```python
from build123d import *

# Parameters (mm, degrees)
SKETCH1_W           = 550
SKETCH1_H           = 300
BOSS_EXTRUDE1_DEPTH = 200
SHELL1_T            = -1.5
SKETCH2_W           = 550
SKETCH2_H           = 300
BOSS_EXTRUDE2_DEPTH = 1
SKETCH3_W           = 530
SKETCH3_H           = 280
SKETCH3_W_2         = 526
SKETCH3_H_2         = 276
SKETCH3_W_3         = 24
SKETCH3_H_3         = 80
CUT_EXTRUDE1_DEPTH  = 0.5
SKETCH5_R           = 11
SKETCH5_W           = 92
SKETCH5_H           = 45
CUT_EXTRUDE2_DEPTH  = 0.5


with BuildPart() as part:
    # Sketch1 → Boss-Extrude1 (new body)
    with BuildSketch(Plane.XY):
        with Locations((275, 150)):
            Rectangle(SKETCH1_W, SKETCH1_H)
    extrude(amount=BOSS_EXTRUDE1_DEPTH)

    # Shell1
    shell1_openings = [part.faces().sort_by_distance(p)[0] for p in [
        (275, 150, 200),
    ]]
    offset(amount=SHELL1_T, openings=shell1_openings, kind=Kind.INTERSECTION)

    # Sketch2 → Boss-Extrude2 (add)
    with BuildSketch(Plane.XY.offset(200)):
        with Locations((275, 150)):
            Rectangle(SKETCH2_W, SKETCH2_H)
    extrude(amount=BOSS_EXTRUDE2_DEPTH)

    # Sketch3 → Cut-Extrude1 (cut)
    # profile 1 of 2: a face of its own
    with BuildSketch(Plane.XY.offset(201)):
        with Locations((275, 150)):
            Rectangle(SKETCH3_W, SKETCH3_H)
        with Locations((275, 150)):
            Rectangle(SKETCH3_W_2, SKETCH3_H_2, mode=Mode.SUBTRACT)
    # profile 2 of 2: a face of its own
    with BuildSketch(Plane.XY.offset(201)):
        with Locations((511, 150)):
            Rectangle(SKETCH3_W_3, SKETCH3_H_3)
    extrude(amount=-CUT_EXTRUDE1_DEPTH, mode=Mode.SUBTRACT)

    # Sketch5 → Cut-Extrude2 (cut)
    with BuildSketch(Plane(origin=(550, 0, 0), x_dir=(0, 0, -1), z_dir=(1, 0, 0))):
        with Locations((-143, 110)):
            Circle(SKETCH5_R)
        with Locations((-58, 110)):
            Circle(SKETCH5_R)
        with Locations((-100.5, 217.5)):
            Rectangle(SKETCH5_W, SKETCH5_H)
    extrude(amount=-CUT_EXTRUDE2_DEPTH, mode=Mode.SUBTRACT)


solid = part.part
```
The model under review builds one solid part; all positions refer to its coordinate system, in mm. A direction names the side the tool comes from. Round coordinates to 2 decimals unless told otherwise and drop trailing zeros. Write each loop counter-clockwise with the first axis right and the second up, starting at its lowest first coordinate (ties: lowest second). Pieces come first, ordered by that corner, then holes. Notation, with made-up numbers: (-2.75, 4) - (22.25, 4) arc R22 cw to (22.25, 29) - close; hole circle Ø4 at (18, 36.5). An arc over 180 degrees is marked (long way). Use one line per item in the form item = value.
Q1. For line 1 (Y direction, x = 549.8, z = 58); line 2 (Z direction, x = 52.5, y = 51.5); line 3 (X direction, y = 115, z = 127.5), list the stretches that pass through material, from the lowest coordinate up. Write a range as [from, to].
Answer key:
line_1 = [0, 99], [121, 195], [240, 300]
line_2 = [0, 1.5], [200, 201]
line_3 = [0, 1.5], [548.5, 550]
Q2. Draft analysis for pull direction Z (two halves, no side actions). For faces 1 (the flat face through (548.5, 148, 99)), 2 (the flat face through (192, 6, 201)), 3 (the flat face through (271, 152, 0)), state which applies: +Z half, -Z half, draft (parallel to the pull), parting line (faces both ways), or undercut.
Answer key:
face_1 = undercut
face_2 = +Z half
face_3 = -Z half
Q3. Consider section C-C (z = 171). State the section outline as (x, y) points.
Answer key:
outline = (0, 0) - (550, 0) - (550, 300) - (0, 300) - close; hole (1.5, 1.5) - (548.5, 1.5) - (548.5, 298.5) - (1.5, 298.5) - close
Q4. Insertion check: pin 1 Ø13 at (y, z) = (110, 143) entering from -X; pin 2 Ø13.5 at (y, z) = (227, 83.5) entering from +X. Each pin has a flat end and moves straight along its axis. Give the tip position at first contact, or say it passes through.
Answer key:
pin_1 = 0
pin_2 = 549.5
Q5. Tool access review of faces 4 (the flat face through (511, 151, 200.5)), 5 (the flat face through (0, 148, 99)), 6 (the flat face through (549.5, 218, 101)), 7 (the flat face through (271, 0, 99)), 8 (the flat face through (271, 298.5, 99)): name each direction out of +Z, -Z, +X, -X, +Y, -Y from which nothing blocks a thin tool from reaching the whole face with its end or side.
Answer key:
face_4 = +Z
face_5 = +Z, -Z, -X, +Y, -Y
face_6 = +X
face_7 = +Z, -Z, +X, -X, -Y
face_8 = none
Q6. Consider section A-A (z = 77). State the section outline as (x, y) points, and give its area (3 significant figures).
Answer key:
outline = (0, 0) - (550, 0) - (550, 195) - (549.5, 195) - (549.5, 240) - (550, 240) - (550, 300) - (0, 300) - close; hole (1.5, 1.5) - (548.5, 1.5) - (548.5, 298.5) - (1.5, 298.5) - close
area = 2,520 mm2
Q7. Consider section B-B (x = 221). State the section outline as (y, z) points, and give its area (3 significant figures).
Answer key:
outline = (0, 0) - (300, 0) - (300, 201) - (290, 201) - (290, 200.5) - (288, 200.5) - (288, 201) - (12, 201) - (12, 200.5) - (10, 200.5) - (10, 201) - (0, 201) - close; hole (1.5, 1.5) - (298.5, 1.5) - (298.5, 200) - (1.5, 200) - close
area = 1,340 mm2
